from build123d import *

# Parameters (mm, degrees)
SKETCH_1_W         = 50
SKETCH_1_H         = 16
EXTRUDE_1_DEPTH    = 1.5
HOLE_WIZARD_M3_1_D = 2.5
CHAMFER_1_SIZE     = 1


with BuildPart() as part:
    # 草图1 → 凸台-拉伸1 (new, symmetric)
    with BuildSketch(Plane.XY):
        Rectangle(SKETCH_1_W, SKETCH_1_H)
    extrude(amount=EXTRUDE_1_DEPTH, both=True)

    # M3 螺纹孔1 (through all)
    with Locations(Plane(origin=(0, 0, -1.5), x_dir=(-1, 0, 0), z_dir=(0, 0, -1))):
        with Locations((12.5, 0), (-12.5, 0)):
            Hole(HOLE_WIZARD_M3_1_D / 2)

    # 倒角1
    chamfer_1_edges = [part.edges().sort_by_distance(p)[0] for p in [
        (25, -8, 0),
        (-25, -8, 0),
        (-25, 8, 0),
        (25, 8, 0),
    ]]
    chamfer(chamfer_1_edges, length=CHAMFER_1_SIZE)


solid = part.part
Check sheet for the modelled part. Datum: model origin and axes. Units: mm. Give positions to 0.01 mm unless a question says otherwise; leave off trailing zeros. Write each loop counter-clockwise with the first axis right and the second up, starting at its lowest first coordinate (ties: lowest second). Pieces come first, ordered by that corner, then holes. Notation, with made-up numbers: (55.25, 20) -> (89.25, 20) arc R16 ccw to (89.25, 27) -> close; hole circle Ø7 at (83, -36.75). An arc over 180 degrees is marked (long way). One line per item, written item: value. Start each with the question number.
Item 1: Material ranges on probe 1 along Y at (x, z) = (12.5, -0.15); probe 2 along X at (y, z) = (-0.5, 1.3); probe 3 along X at (y, z) = (0.75, -0.15), recorded low to high. Write a range as from..to.
Item 2: Section check A-A on y = 0. Record the cut outline in (x, z).
Item 3: Section check B-B on x = 12.5. Record the cut outline in (y, z).
Item 4: Draft check along Y on faces 1 (the flat face through (24.5, 7.5, 0)), 2 (the cylindrical face through (-13.75, 0.05, 0.02)), 3 (the flat face through (-24.5, -7.5, 0)). Enter one of: +Y half, -Y half, draft (parallel to the pull), parting line (faces both ways), or undercut.
Results list:
1. probe 1: -8..-1.25, 1.25..8
1. probe 2: -25..-13.65, -11.35..11.35, 13.65..25
1. probe 3: -25..-13.5, -11.5..11.5, 13.5..25
2. outline: (-25, -1.5) -> (-13.75, -1.5) -> (-13.75, 1.5) -> (-25, 1.5) -> close; (-11.25, -1.5) -> (11.25, -1.5) -> (11.25, 1.5) -> (-11.25, 1.5) -> close; (13.75, -1.5) -> (25, -1.5) -> (25, 1.5) -> (13.75, 1.5) -> close
3. outline: (-8, -1.5) -> (-1.25, -1.5) -> (-1.25, 1.5) -> (-8, 1.5) -> close; (1.25, -1.5) -> (8, -1.5) -> (8, 1.5) -> (1.25, 1.5) -> close
4. face 1: +Y half
4. face 2: undercut
4. face 3: -Y half
